from build123d import *

# Parameters (mm, degrees)
BOSS_EXTRUDE1_DEPTH = 7.5
SKETCH4_R           = 20.03
SKETCH4_R_2         = 9
CUT_EXTRUDE1_DEPTH  = 0.9375
CUT_EXTRUDE1_DRAFT  = -60
CHAMFER2_SIZE       = 0.666666667
SKETCH9_R           = 8.815
SKETCH9_R_2         = 3
CUT_EXTRUDE2_DEPTH  = 15


with BuildPart() as part:
    # Sketch3 → Boss-Extrude1 (new body)
    with BuildSketch(Plane(origin=(0, 0, 0), x_dir=(0, 0, -1), z_dir=(1, 0, 0))):
        Polygon((9, 5.196152423), (0, 10.392304845), (-9, 5.196152423), (-9, -5.196152423), (0, -10.392304845), (9, -5.196152423), align=None)
    extrude(amount=BOSS_EXTRUDE1_DEPTH)


with BuildPart() as cut_extrude1_tool:
    # Sketch4 → Cut-Extrude1 (with draft: the straight prism first)
    with BuildSketch(Plane.ZY):
        Circle(SKETCH4_R)
        Circle(SKETCH4_R_2, mode=Mode.SUBTRACT)
    extrude(amount=-CUT_EXTRUDE1_DEPTH)
    # Cut-Extrude1: the draft: its side faces are tilted about the plane it starts from
    cut_extrude1_sides = [cut_extrude1_tool.faces().sort_by_distance(p)[0] for p in [
        (0.46875, 0, -20.03),
        (0.46875, 0, -9),
    ]]
    draft(cut_extrude1_sides, Plane.ZY, CUT_EXTRUDE1_DRAFT)


with BuildPart() as part_1:
    add(part.part)

    # Cut-Extrude1: cut by cut_extrude1_tool
    add(cut_extrude1_tool.part, mode=Mode.SUBTRACT)

    # Sketch5 → Revolve1 (revolve)
    with BuildSketch(Plane.XY, mode=Mode.PRIVATE) as revolve1_sk:
        with BuildLine():
            Line((8.35, 6), (87.5, 6))
            Line((87.5, 6), (87.5, 0))
            Line((87.5, 0), (7.5, 0))
            Line((7.5, 0), (7.5, 6.85))
            ThreePointArc((7.5, 6.85), (7.748959236, 6.248959236), (8.35, 6))
        make_face()
    revolve(revolve1_sk.sketch.rotate(Axis((7.5, 0, 0), (1, 0, 0)), 90), axis=Axis((7.5, 0, 0), (1, 0, 0)))

    # Chamfer2
    chamfer2_edges = [part_1.edges().sort_by_distance(p)[0] for p in [
        (87.5, 0, -6),
    ]]
    chamfer(chamfer2_edges, length=CHAMFER2_SIZE)

    # Sketch7 → Cut-Revolve1 (revolve, cut)
    with BuildSketch(Plane.XY, mode=Mode.PRIVATE) as cut_revolve1_sk:
        Polygon((7.5, 8.215), (6.9, 8.815), (6.9, 20.03), (7.5, 20.03), align=None)
    revolve(cut_revolve1_sk.sketch.rotate(Axis((0, 0, 0), (1, 0, 0)), 90), axis=Axis((0, 0, 0), (1, 0, 0)), mode=Mode.SUBTRACT)

    # Sketch9 → Cut-Extrude2 (cut)
    with BuildSketch(Plane(origin=(87.5, 0, 0), x_dir=(0, 0, -1), z_dir=(1, 0, 0))):
        Circle(SKETCH9_R)
        Circle(SKETCH9_R_2, mode=Mode.SUBTRACT)
    extrude(amount=-CUT_EXTRUDE2_DEPTH, mode=Mode.SUBTRACT)


solid = part_1.part
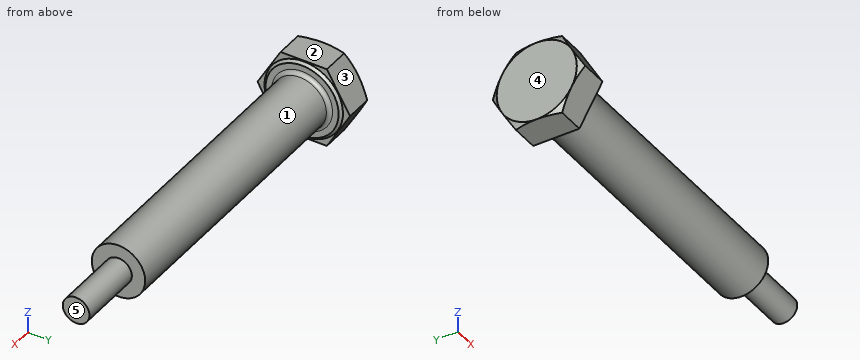
Work out the finished part from the listing and answer in its coordinate system (mm). Face numbers are marked on the shaded views. A direction names the side the tool comes from. Coordinates: 2 decimals unless noted, no trailing zeros. Write each loop counter-clockwise with the first axis right and the second up, starting at its lowest first coordinate (ties: lowest second). Pieces come first, ordered by that corner, then holes. Notation, with made-up numbers: M 28,-15 L 60,-15 A15 cw 60,-9 Z; hole C 47.25,69 d5. An arc over 180 degrees is marked long. Answer as CSV lines item,"result". Start each with the question number.
Item 1: Section A-A on x = 61.5 is taken. Write down the section's boundary in (y, z).
Item 2: Section B-B on x = 74.5 is taken. Write down the section's boundary in (y, z).
Item 3: Flat-ended cylindrical pins translate along their axes: P1, Ø5, axis at y = -1, z = -5.5, coming from the -X side; P2, Ø3, axis at x = 66.5, z = 1.5, coming from the +Y side; P3, Ø3, axis at x = 27, y = 2, coming from the +Z side; P4, Ø12, axis at x = 39.5, y = 5, coming from the -Z side. Find the tip coordinate at first contact, or state that the pin passes through.
Item 4: A tool of negligible diameter and unlimited length cuts with its end or side. For the marked faces 1 and 2, from which of +Z, -Z, +X, -X, +Y, -Y can it reach the whole face along a straight path? Write none if from no direction.
Item 5: Determine the mould class of the marked faces 3, 4 and 5 for opening direction X: released by +X, released by -X, zero draft, split by the parting line, or undercut.
Item 6: Consider L1, parallel to X at y = 2, z = 2.75; L2, parallel to X at y = -7, z = 0.5; L3, parallel to Z at x = 44.5, y = 0.25. Determine where each line is inside the solid, lowest interval first.
Checks:
1,outline,"C 0,0 d12"
2,outline,"C 0,0 d6"
3,P1,"stops at x = 0"
3,P2,"stops at y = 6"
3,P3,"stops at z = 5.98"
3,P4,"stops at z = -6"
4,face 1,"+X"
4,face 2,"+Z, +X, -X, +Y, -Y"
5,face 3,"zero draft"
5,face 4,"released by -X"
5,face 5,"released by +X"
6,L1,"x = 0 to 72.5"
6,L2,"x = 0 to 7.5"
6,L3,"z = -5.99 to 5.99"
